Design review of the part built by this model. Coordinates are the model's own, in mm. Face numbers are marked on the shaded views. Give positions to 0.01 mm unless a question says otherwise; leave off trailing zeros. Order: outer loops, then holes, each group sorted by start corner. A loop starts at its lowest first (then second) coordinate and runs counter-clockwise, first axis right, second up. Notation, with made-up numbers: M 30.25,76.25 L 35.25,76.25 A18 ccw 35.25,106.25 Z; hole C 49,-0.75 d6. An arc over 180 degrees is marked long. Answer as a JSON object with one key per item and string values.
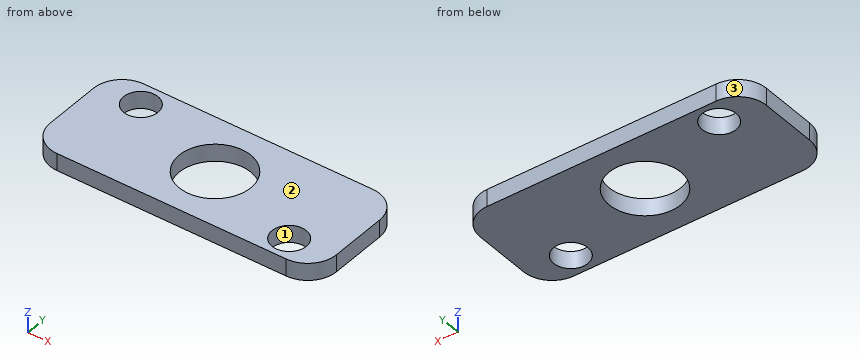
from build123d import *

# Parameters (mm, degrees)
SKETCH_1_R      = 3
SKETCH_1_R_2    = 6.25
EXTRUDE_1_DEPTH = 3


with BuildPart() as part:
    # 草图1 → 凸台-拉伸1 (new body)
    with BuildSketch(Plane.XY.offset(1.5)):
        with BuildLine():
            Line((-20, -10), (20, -10))
            ThreePointArc((20, -10), (23.535533906, -8.535533906), (25, -5))
            Line((25, -5), (25, 5))
            ThreePointArc((25, 5), (23.535533906, 8.535533906), (20, 10))
            Line((20, 10), (-20, 10))
            ThreePointArc((-20, 10), (-23.535533906, 8.535533906), (-25, 5))
            Line((-25, 5), (-25, -5))
            ThreePointArc((-25, -5), (-23.535533906, -8.535533906), (-20, -10))
        make_face()
        with Locations(Location((-17.5, 6, 0), (0, 0, 180))):
            Circle(SKETCH_1_R, mode=Mode.SUBTRACT)
        with Locations(Location((17.5, -6, 0), (0, 0, 180))):
            Circle(SKETCH_1_R, mode=Mode.SUBTRACT)
        with Locations(Location((0, 0, 0), (0, 0, 180))):
            Circle(SKETCH_1_R_2, mode=Mode.SUBTRACT)
    extrude(amount=-EXTRUDE_1_DEPTH)


solid = part.part
(1) Draft analysis for pull direction Y (two halves, no side actions). For the marked faces 1, 2 and 3, state which applies: +Y half, -Y half, draft (parallel to the pull), parting line (faces both ways), or undercut.
Checked values:
{"face 1": "undercut", "face 2": "draft", "face 3": "+Y half"}
(2) To check wall thickness, follow L1, parallel to Y at x = 17.5, z = 0.75; L2, parallel to X at y = 4.5, z = -0.65; L3, parallel to X at y = -4.5, z = 0.3. State the ranges of each line that lie inside material, in increasing order. Write a range as from..to.
Checked values:
{"L1": "y = -10..-9, -3..10", "L2": "x = -25..-20.1, -14.9..-4.34, 4.34..25", "L3": "x = -25..-4.34, 4.34..14.9, 20.1..25"}
(3) We need section C-C (y = 0.5). Write out the cut boundary in (x, z), plus the area to 3 significant figures.
Checked values:
{"outline": "M -25,-1.5 L -6.23,-1.5 L -6.23,1.5 L -25,1.5 Z; M 6.23,-1.5 L 25,-1.5 L 25,1.5 L 6.23,1.5 Z", "area": "113 mm^2"}
(4) We need section A-A (x = 0). Write out the cut boundary in (y, z), plus the area to 3 significant figures.
Checked values:
{"outline": "M -10,-1.5 L -6.25,-1.5 L -6.25,1.5 L -10,1.5 Z; M 6.25,-1.5 L 10,-1.5 L 10,1.5 L 6.25,1.5 Z", "area": "22.5 mm^2"}
(5) We need section B-B (z = 0.8). Write out the cut boundary in (x, y).
Checked values:
{"outline": "M -25,-5 A5 ccw -20,-10 L 20,-10 A5 ccw 25,-5 L 25,5 A5 ccw 20,10 L -20,10 A5 ccw -25,5 Z; hole C -17.5,6 d6; hole C 0,0 d12.5; hole C 17.5,-6 d6"}
